Can you work these out from the model? Positions are in its coordinate system, mm. A direction names the side the tool comes from. Round coordinates to 2 decimals unless told otherwise and drop trailing zeros. Loops run counter-clockwise (first coordinate to the right, second up) from the corner with the lowest first, then second, coordinate; pieces in that order, holes last.
from build123d import *

# Parameters (mm, degrees)
BASE_PLATE_SKETCH_W        = 100
BASE_PLATE_SKETCH_H        = 70
BASE_PLATE_DEPTH           = 30
SEMICIRCULAR_NOTCH_DEPTH   = 30
UPRIGHT_WALL_SKETCH_W      = 50
UPRIGHT_WALL_SKETCH_H      = 70
UPRIGHT_WALL_DEPTH         = 20
HALF_ROUND_BOSS_SKETCH_R   = 20
HALF_ROUND_BOSS_SKETCH_R_2 = 10
HALF_ROUND_BOSS_DEPTH      = 40


with BuildPart() as part:
    # Base Plate Sketch → Base Plate (new body)
    with BuildSketch(Plane.XY):
        with Locations((50, 35)):
            Rectangle(BASE_PLATE_SKETCH_W, BASE_PLATE_SKETCH_H)
    extrude(amount=BASE_PLATE_DEPTH)

    # Notch Sketch → Semicircular Notch (cut)
    with BuildSketch(Plane.XY.offset(30)):
        with BuildLine():
            Line((0, 45), (0, 25))
            ThreePointArc((0, 25), (10, 35), (0, 45))
        make_face()
    extrude(amount=-SEMICIRCULAR_NOTCH_DEPTH, mode=Mode.SUBTRACT)

    # Upright Wall Sketch → Upright Wall (add)
    with BuildSketch(Plane(origin=(100, 0, 0), x_dir=(0, 0, -1), z_dir=(1, 0, 0))):
        with Locations((-55, 35)):
            Rectangle(UPRIGHT_WALL_SKETCH_W, UPRIGHT_WALL_SKETCH_H)
    extrude(amount=-UPRIGHT_WALL_DEPTH)

    # Half-Round Boss Sketch → Half-Round Boss (add)
    with BuildSketch(Plane.ZY.offset(-80)):
        with Locations(Location((55, 35, 0), (0, 0, 180))):
            Circle(HALF_ROUND_BOSS_SKETCH_R)
        with Locations((55, 35)):
            Circle(HALF_ROUND_BOSS_SKETCH_R_2, mode=Mode.SUBTRACT)
    extrude(amount=HALF_ROUND_BOSS_DEPTH)


solid = part.part
(1) Will these pins go through, and if not, where does the flat tip stop? P1, Ø3, axis at y = 44, z = 36.5, coming from the -X side; P2, Ø4, axis at x = 88, z = 57.5, coming from the -Y side; P3, Ø5, axis at x = 65.5, z = 50, coming from the +Y side; P4, Ø10, axis at x = 25.5, y = 35, coming from the +Z side.
Worked answers:
P1: stops at x = 40
P2: stops at y = 0
P3: stops at y = 54.84
P4: stops at z = 30
(2) If we section it at B-B, the plane z = 55: List the corners of the cut face in (x, y) for me, then the cut area to 3 significant figures.
Worked answers:
outline: (40, 15) - (80, 15) - (80, 0) - (100, 0) - (100, 70) - (80, 70) - (80, 55) - (40, 55) - (40, 45) - (80, 45) - (80, 25) - (40, 25) - close
area: 2,200 mm2
(3) If we section it at D-D, the plane y = 11.5: List the corners of the cut face in (x, z) for me.
Worked answers:
outline: (0, 0) - (100, 0) - (100, 80) - (80, 80) - (80, 30) - (0, 30) - close
(4) If we section it at A-A, the plane x = 51.5: List the corners of the cut face in (y, z) for me, then the cut area to 3 significant figures.
Worked answers:
outline: (0, 0) - (70, 0) - (70, 30) - (0, 30) - close; circle Ø40 at (35, 55); hole circle Ø20 at (35, 55)
area: 3,040 mm2
(5) If we section it at C-C, the plane y = 35: List the corners of the cut face in (x, z) for me.
Worked answers:
outline: (10, 0) - (100, 0) - (100, 80) - (80, 80) - (80, 75) - (40, 75) - (40, 65) - (80, 65) - (80, 45) - (40, 45) - (40, 35) - (80, 35) - (80, 30) - (10, 30) - close
(6) For faces 1 (the flat face through (39, 35, 30)), 2 (the flat face through (80, 35, 78)), 3 (the flat face through (40, 30, 64)), which set-ups out of +Z, -Z, +X, -X, +Y, -Y let a thin tool reach every point of the face, with its end or its side?
Worked answers:
face 1: -X, +Y, -Y
face 2: -X
face 3: +Z, -X, +Y, -Y
(7) If I drill on line 1 (Y direction, x = 70, z = 55); line 2 (X direction, y = 7, z = 68.5); line 3 (Z direction, x = 23.5, y = 60), over which ranges is the centre line in solid material (lowest first)?
Worked answers:
line 1: y = 15 to 25, 45 to 55
line 2: x = 80 to 100
line 3: z = 0 to 30
(8) If we mould it in two halves opening along Z, with no side actions, what happens to faces 4 (the flat face through (100, 35, 41)), 5 (the flat face through (90, 35, 80)), 6 (the flat face through (49, 35, 0)), 7 (the flat face through (80, 35, 55))? For each: released by +Z, released by -Z, zero draft, split by the parting line, or undercut.
Worked answers:
face 4: zero draft
face 5: released by +Z
face 6: released by -Z
face 7: undercut
